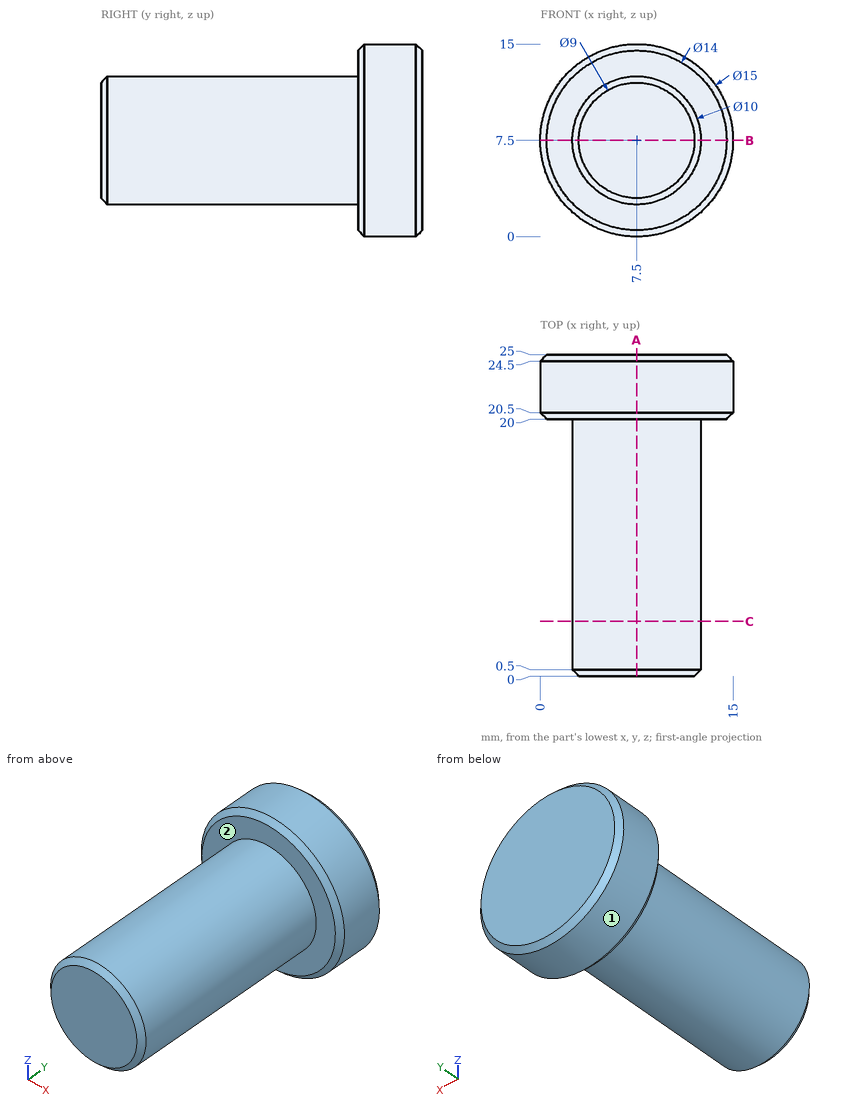
Here's the drawing with two shaded views (mm, measured from the low corner). I have some questions. A direction names the side the tool comes from. Coordinates: 2 decimals unless noted, no trailing zeros. Loops run counter-clockwise (first coordinate to the right, second up) from the corner with the lowest first, then second, coordinate; pieces in that order, holes last. Notation, with made-up numbers: (56, 6.5) -> (60, 6.5) arc R11 cw to (60, 14.5) -> close; hole circle Ø11 at (68, -19). An arc over 180 degrees is marked (long way). Put each result on its own line as item: value. Start each with the question number.
Q1. I want a section at A-A (x = 7.5). Write out the boundary of the cut face in (y, z), plus the area to 3 significant figures.
Q2. For the marked faces 1 and 2, which set-ups out of +Z, -Z, +X, -X, +Y, -Y let a thin tool reach every point of the face, with its end or its side?
Q3. If I drill on line 1 (Y direction, x = 9.75, z = 1); line 2 (X direction, y = 16.75, z = 7.75); line 3 (X direction, y = 8, z = 4.5), over which ranges is the centre line in solid material (lowest first)? Write a range as [from, to].
Q4. I want a section at B-B (z = 7.5). Write out the boundary of the cut face in (x, y).
Q5. I want a section at C-C (y = 4.25). Write out the boundary of the cut face in (x, z).
Q6. I'm going to push flat-ended pins straight in: P1, Ø5, axis at x = 1.5, y = 10, coming from the -Z side; P2, Ø4, axis at y = 15.5, z = 8.5, coming from the +X side; P3, Ø4, axis at x = 2, y = 16.5, coming from the +Z side. Where does each tip first touch, or does it pass through?
Taken from the geometry:
1. outline: (0, 3) -> (0.5, 2.5) -> (20, 2.5) -> (20, 0.5) -> (20.5, 0) -> (24.5, 0) -> (25, 0.5) -> (25, 14.5) -> (24.5, 15) -> (20.5, 15) -> (20, 14.5) -> (20, 12.5) -> (0.5, 12.5) -> (0, 12) -> close
1. area: 274 mm2
2. face 1: +Y, -Y
2. face 2: -Y
3. line 1: y = [20, 25]
3. line 2: x = [2.51, 12.49]
3. line 3: x = [3.5, 11.5]
4. outline: (0, 20.5) -> (0.5, 20) -> (2.5, 20) -> (2.5, 0.5) -> (3, 0) -> (12, 0) -> (12.5, 0.5) -> (12.5, 20) -> (14.5, 20) -> (15, 20.5) -> (15, 24.5) -> (14.5, 25) -> (0.5, 25) -> (0, 24.5) -> close
5. outline: circle Ø10 at (7.5, 7.5)
6. P1: stops at z = 3.93
6. P2: stops at x = 12.5
6. P3: stops at z = 11.07
